```python
from build123d import *

# Parameters (mm, degrees)
SKETCH_1_W               = 90
SKETCH_1_H               = 90
EXTRUDE_1_DEPTH          = 10
FILLET_1_R               = 10
SKETCH_2_R               = 4.5
SKETCH_2_R_2             = 4.53
CUT_EXTRUDE_1_DEPTH      = 65.420493634
SKETCH_3_R               = 37.5
EXTRUDE_2_DEPTH          = 5
SKETCH_4_R               = 17.5
EXTRUDE_3_DEPTH          = 7
SKETCH_5_R               = 15
CUT_EXTRUDE_2_DEPTH      = 68.334983478
SKETCH_6_R               = 5.5
CUT_EXTRUDE_3_DEPTH      = 7
SKETCH_7_R               = 3.5
CUT_EXTRUDE_4_DEPTH      = 66.383484153
PATTERN_CIRCULAR_1_COUNT = 3
FILLET_2_R               = 2
CHAMFER_1_SIZE           = 1


with BuildPart() as part:
    # 草图1 → 凸台-拉伸1 (new body)
    with BuildSketch(Plane.XY):
        Rectangle(SKETCH_1_W, SKETCH_1_H)
    extrude(amount=EXTRUDE_1_DEPTH)

    # 圆角1
    fillet_1_edges = [part.edges().sort_by_distance(p)[0] for p in [
        (45, -45, 5),
        (-45, -45, 5),
        (-45, 45, 5),
        (45, 45, 5),
    ]]
    fillet(fillet_1_edges, radius=FILLET_1_R)

    # 草图2 → 切除-拉伸1 (cut, through all)
    with BuildSketch(Plane.XY.offset(10)):
        with Locations((-34, 34)):
            Circle(SKETCH_2_R)
        with Locations((34, 34)):
            Circle(SKETCH_2_R)
        with Locations((-34, -34)):
            Circle(SKETCH_2_R)
        with Locations((34, -34)):
            Circle(SKETCH_2_R_2)
    extrude(amount=-CUT_EXTRUDE_1_DEPTH, mode=Mode.SUBTRACT)

    # 草图3 → 凸台-拉伸2 (add)
    with BuildSketch(Plane.XY.offset(10)):
        Circle(SKETCH_3_R)
    extrude(amount=EXTRUDE_2_DEPTH)

    # 草图4 → 凸台-拉伸3 (add)
    with BuildSketch(Plane(origin=(0, 0, 0), x_dir=(-1, 0, 0), z_dir=(0, 0, -1))):
        with Locations(Location((0, 0, 0), (0, 0, 180))):
            Circle(SKETCH_4_R)
    extrude(amount=EXTRUDE_3_DEPTH)

    # 草图5 → 切除-拉伸2 (cut, through all)
    with BuildSketch(Plane.XY.offset(15)):
        Circle(SKETCH_5_R)
    extrude(amount=-CUT_EXTRUDE_2_DEPTH, mode=Mode.SUBTRACT)

    # 草图6 → 切除-拉伸3 (cut)
    with BuildSketch(Plane.XY.offset(15)):
        with Locations((0, 27)):
            Circle(SKETCH_6_R)
    cut_extrude_3 = extrude(amount=-CUT_EXTRUDE_3_DEPTH, mode=Mode.SUBTRACT)

    # 草图7 → 切除-拉伸4 (cut, through all)
    with BuildSketch(Plane.XY.offset(8)):
        with Locations((0, 27)):
            Circle(SKETCH_7_R)
    cut_extrude_4 = extrude(amount=-CUT_EXTRUDE_4_DEPTH, mode=Mode.SUBTRACT)

    # 阵列(圆周)1: 切除-拉伸3, 切除-拉伸4 ×3 about axis
    pattern_circular_1_axis = Axis((0, 0, 0), (0, 0, 1))
    add([cut_extrude_3.rotate(pattern_circular_1_axis, i * 360 / PATTERN_CIRCULAR_1_COUNT) for i in range(1, PATTERN_CIRCULAR_1_COUNT)], mode=Mode.SUBTRACT)
    add([cut_extrude_4.rotate(pattern_circular_1_axis, i * 360 / PATTERN_CIRCULAR_1_COUNT) for i in range(1, PATTERN_CIRCULAR_1_COUNT)], mode=Mode.SUBTRACT)

    # 圆角2
    fillet_2_edges = [part.edges().sort_by_distance(p)[0] for p in [
        (-37.5, 0, 10),
    ]]
    fillet(fillet_2_edges, radius=FILLET_2_R)

    # 倒角1
    chamfer_1_edges = [part.edges().sort_by_distance(p)[0] for p in [
        (-37.5, 0, 15),
        (-17.5, 0, -7),
        (-15, 0, 15),
    ]]
    chamfer(chamfer_1_edges, length=CHAMFER_1_SIZE)


solid = part.part
```
CAD build for the part. Positions are in the model's coordinates, mm. A direction names the side the tool comes from. Coordinates: 2 decimals unless noted, no trailing zeros. Order: outer loops, then holes, each group sorted by start corner. A loop starts at its lowest first (then second) coordinate and runs counter-clockwise, first axis right, second up. Notation, with made-up numbers: (36.25, 1) -> (84.25, 1) arc R31 cw to (84.25, 36) -> close; hole circle Ø8 at (27, 57). An arc over 180 degrees is marked (long way). Use one line per item in the form item = value. Start each with the question number.
1) Drop flat-ended pins along their axis: pin 1 (14.5 mm diameter, centred on x = -34, y = -34, fed in from +Z); pin 2 (8 mm diameter, centred on x = 0, y = 27, fed in from -Z); pin 3 (10 mm diameter, centred on x = 23.38, y = -13.5, fed in from +Z); pin 4 (5.5 mm diameter, centred on x = -2.5, y = 29, fed in from +Z). Give the stop position or say it passes through.
2) Tool access for faces 4 (the flat face through (-1, 21, 0)), 5 (the flat face through (-41, 1, 10)), 6 (the cylindrical face through (36.435, -30.18, 5.07)): list every direction of +Z, -Z, +X, -X, +Y, -Y with a clear straight run to the whole face (end or side of a thin tool).
3) Drill centre lines: L1, parallel to Y at x = -34, z = 3.25; L2, parallel to Y at x = 0, z = 2.5; L3, parallel to Z at x = -15, y = -11.5. Where is each one in solid material? Low to high. Write a range as [from, to].
4) Band-saw the part on B-B on y = -13.5. State how many separate pieces and enclosed holes the cut face has, then the cut area to 3 significant figures.
5) Band-saw the part on A-A on y = 0. Give the cut face in (x, z).
6) Pull direction X, two halves, no side cores. Call faces 1 (the cylindrical face through (-24.57, -18.87, 11.55)), 2 (the cylindrical face through (42.15, 41.99, 5.07)), 3 (the flat face through (-45, 0, 5)): +X half, -X half, draft (parallel to the pull), parting line (faces both ways), or undercut.
Entries:
q1.pin_1 = 10
q1.pin_2 = 0
q1.pin_3 = 8
q1.pin_4 = 15
q2.face_4 = -Z
q2.face_5 = +Z
q2.face_6 = +Z, -Z
q3.L1 = [-45, -38.5], [-29.5, 29.5], [38.5, 45]
q3.L2 = [-45, -15], [15, 23.5], [30.5, 45]
q3.L3 = [0, 15]
q4.separate_pieces = 4
q4.enclosed_holes = 0
q4.area = 849 mm2
q5.outline = (-45, 0) -> (-17.5, 0) -> (-17.5, -6) -> (-16.5, -7) -> (-15, -7) -> (-15, 14) -> (-16, 15) -> (-36.5, 15) -> (-37.5, 14) -> (-37.5, 12) arc R2 cw to (-39.5, 10) -> (-45, 10) -> close; (15, -7) -> (16.5, -7) -> (17.5, -6) -> (17.5, 0) -> (45, 0) -> (45, 10) -> (39.5, 10) arc R2 cw to (37.5, 12) -> (37.5, 14) -> (36.5, 15) -> (16, 15) -> (15, 14) -> close
q6.face_1 = undercut
q6.face_2 = +X half
q6.face_3 = -X half
